from build123d import *

# Parameters (mm, degrees)
SKETCH_1_W      = 645
SKETCH_1_H      = 596
EXTRUDE_1_DEPTH = 22
SHELL_1_T       = -2
SKETCH_2_W      = 645
SKETCH_2_H      = 596
SKETCH_2_W_2    = 605
SKETCH_2_H_2    = 556
EXTRUDE_2_DEPTH = 2


with BuildPart() as part:
    # 草图1 → 凸台-拉伸1 (new body)
    with BuildSketch(Plane.XY):
        with Locations((322.5, 298)):
            Rectangle(SKETCH_1_W, SKETCH_1_H)
    extrude(amount=EXTRUDE_1_DEPTH)

    # 抽壳1
    shell_1_openings = [part.faces().sort_by_distance(p)[0] for p in [
        (322.5, 298, 22),
    ]]
    offset(amount=SHELL_1_T, openings=shell_1_openings, kind=Kind.INTERSECTION)

    # 草图2 → 凸台-拉伸2 (add)
    with BuildSketch(Plane.XY.offset(22)):
        with Locations((322.5, 298)):
            Rectangle(SKETCH_2_W, SKETCH_2_H)
        with Locations((322.5, 298)):
            Rectangle(SKETCH_2_W_2, SKETCH_2_H_2, mode=Mode.SUBTRACT)
    extrude(amount=-EXTRUDE_2_DEPTH)


solid = part.part
Input: part model. Units: mm. Frame: model coordinates. A direction names the side the tool comes from. Round coordinates to 2 decimals unless told otherwise and drop trailing zeros. Order: outer loops, then holes, each group sorted by start corner. A loop starts at its lowest first (then second) coordinate and runs counter-clockwise, first axis right, second up.
1. Set-up query: faces 4 (the face through (318, 0, 11)), 5 (the face through (318, 2, 11)). Return all of +Z, -Z, +X, -X, +Y, -Y with unobstructed straight access to the full face (end or side cutting, diameter ignored); none if empty.
The answers:
face 4: +Z, -Z, +X, -X, -Y
face 5: none
2. Material intervals for line 1 (X direction, y = 452, z = 17.5); line 2 (Y direction, x = 85, z = 19.5); line 3 (X direction, y = 482, z = 20.5), sorted ascending.
The answers:
line 1: x = 0 to 2, 643 to 645
line 2: y = 0 to 2, 594 to 596
line 3: x = 0 to 20, 625 to 645
3. Mould query, pull axis X, two halves, no side actions, for faces 1 (the face through (318, 594, 11)), 2 (the face through (645, 294, 11)), 3 (the face through (297, 12, 22)). Classes: released by +X, released by -X, zero draft, split by the parting line, or undercut.
The answers:
face 1: undercut
face 2: released by +X
face 3: zero draft
4. Cut plane B-B, the plane y = 207. Output: boundary loops of the cut face in (x, z).
The answers:
outline: (0, 0) - (645, 0) - (645, 22) - (625, 22) - (625, 20) - (643, 20) - (643, 2) - (2, 2) - (2, 20) - (20, 20) - (20, 22) - (0, 22) - close
5. Pin query (flat end, axial travel): P1, Ø6, axis at x = 401, y = 431.5, coming from the +Z side. Return the tip coordinate at first contact, or that it passes through.
The answers:
P1: stops at z = 2
6. Cut plane C-C, the plane x = 353.5. Output: boundary loops of the cut face in (y, z).
The answers:
outline: (0, 0) - (596, 0) - (596, 22) - (576, 22) - (576, 20) - (594, 20) - (594, 2) - (2, 2) - (2, 20) - (20, 20) - (20, 22) - (0, 22) - close
7. Cut plane A-A, the plane z = 10.75. Output: boundary loops of the cut face in (x, y).
The answers:
outline: (0, 0) - (645, 0) - (645, 596) - (0, 596) - close; hole (2, 2) - (643, 2) - (643, 594) - (2, 594) - close
